For this review, take the finished solid that the model builds, in its own axes (mm). Give positions to 0.01 mm unless a question says otherwise; leave off trailing zeros. Write each loop counter-clockwise with the first axis right and the second up, starting at its lowest first coordinate (ties: lowest second). Pieces come first, ordered by that corner, then holes. Notation, with made-up numbers: (-11, 22) -> (41, 22) arc R23 cw to (41, 46) -> close; hole circle Ø4 at (19.25, -33). An arc over 180 degrees is marked (long way). Return JSON: item names as keys, results as strings.
from build123d import *

# Parameters (mm, degrees)
SKETCH1_W           = 20
SKETCH1_H           = 90
SKETCH1_R           = 2.5
BOSS_EXTRUDE1_DEPTH = 5


with BuildPart() as part:
    # Sketch1 → Boss-Extrude1 (new body)
    with BuildSketch(Plane(origin=(0, 0, 0), x_dir=(1, 0, 0), z_dir=(0, 1, 0))):
        Rectangle(SKETCH1_W, SKETCH1_H)
        with Locations(Location((0, 35, 0), (0, 0, 270))):
            Circle(SKETCH1_R, mode=Mode.SUBTRACT)
    extrude(amount=BOSS_EXTRUDE1_DEPTH)


solid = part.part
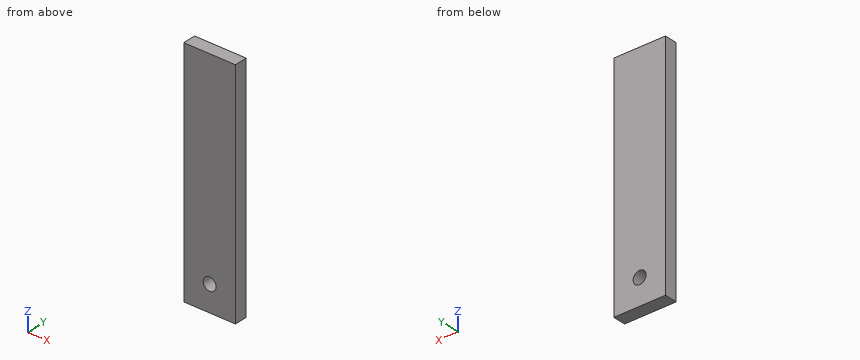
1. Add section B-B, the plane x = 0. State the section outline as (y, z) points.
Results found:
{"outline": "(0, -45) -> (5, -45) -> (5, -37.5) -> (0, -37.5) -> close; (0, -32.5) -> (5, -32.5) -> (5, 45) -> (0, 45) -> close"}
2. For pin 1 (5 mm diameter, centred on x = -1, z = -16.5, fed in from -Y); pin 2 (3 mm diameter, centred on x = 0, z = -35, fed in from -Y), all flat-tipped, find the tip position at first contact; note any pin that passes through.
Results found:
{"pin 1": "stops at y = 0", "pin 2": "passes through"}
3. Add section A-A, the plane z = -35. State the section outline as (x, y) points.
Results found:
{"outline": "(-10, 0) -> (-2.5, 0) -> (-2.5, 5) -> (-10, 5) -> close; (2.5, 0) -> (10, 0) -> (10, 5) -> (2.5, 5) -> close"}
4. To check wall thickness, follow probe 1 along X at (y, z) = (2.6, -35); probe 2 along Z at (x, y) = (-0.75, 3.05); probe 3 along Z at (x, y) = (-1.5, 3.65). State the ranges of each line that lie inside material, in increasing order.
Results found:
{"probe 1": "x = -10 to -2.5, 2.5 to 10", "probe 2": "z = -45 to -37.38, -32.62 to 45", "probe 3": "z = -45 to -37, -33 to 45"}
